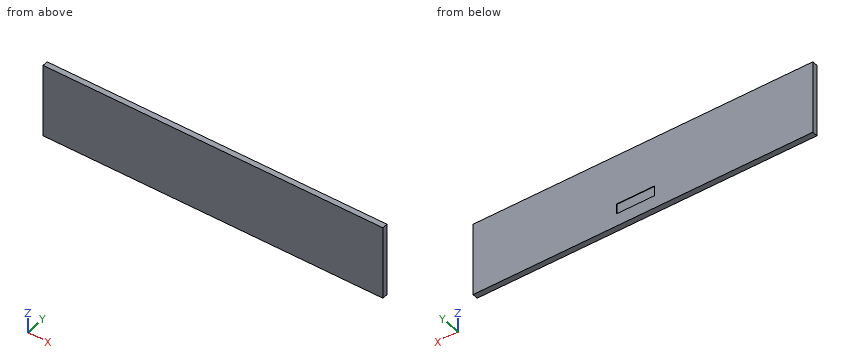
from build123d import *

# Parameters (mm, degrees)
SKETCH_1_W          = 1346
SKETCH_1_H          = 288
EXTRUDE_1_DEPTH     = 20
SHELL_1_T           = -2
SKETCH_2_W          = 1346
SKETCH_2_H          = 288
EXTRUDE_2_DEPTH     = 2
SKETCH_4_W          = 150
SKETCH_4_H          = 40
CUT_EXTRUDE_1_DEPTH = 2


with BuildPart() as part:
    # 草图1 → 凸台-拉伸1 (new body)
    with BuildSketch(Plane(origin=(0, 0, 0), x_dir=(1, 0, 0), z_dir=(0, 1, 0))):
        Rectangle(SKETCH_1_W, SKETCH_1_H)
    extrude(amount=-EXTRUDE_1_DEPTH)

    # 抽壳1
    shell_1_openings = [part.faces().sort_by_distance(p)[0] for p in [
        (0, -20, 0),
    ]]
    offset(amount=SHELL_1_T, openings=shell_1_openings, kind=Kind.INTERSECTION)

    # 草图2 → 凸台-拉伸2 (add)
    with BuildSketch(Plane.XZ.offset(20)):
        Rectangle(SKETCH_2_W, SKETCH_2_H)
    extrude(amount=EXTRUDE_2_DEPTH)

    # 草图4 → 切除-拉伸1 (cut)
    with BuildSketch(Plane(origin=(0, 0, 0), x_dir=(1, 0, 0), z_dir=(0, 1, 0))):
        with Locations((30, 74)):
            Rectangle(SKETCH_4_W, SKETCH_4_H)
    extrude(amount=-CUT_EXTRUDE_1_DEPTH, mode=Mode.SUBTRACT)


solid = part.part
Work out the finished part from the listing and answer in its coordinate system (mm). Give positions to 0.01 mm unless a question says otherwise; leave off trailing zeros. Order: outer loops, then holes, each group sorted by start corner. A loop starts at its lowest first (then second) coordinate and runs counter-clockwise, first axis right, second up. Notation, with made-up numbers: (4, -30.75) -> (60, -30.75) arc R21 ccw to (60, 8.25) -> close; hole circle Ø6 at (15.5, 7.5). An arc over 180 degrees is marked (long way). Answer as a JSON object with one key per item and string values. Group by question number.
1. Section B-B on z = 35 is taken. Determine the outline of the cut face in (x, y), plus the area to 3 significant figures.
2. Consider line 1 along X through (y, z) = (-12.75, 73.5); line 2 along Z through (x, y) = (589.5, -10.25); line 3 along Y through (x, z) = (-508, -84.5). Determine where each line is inside the solid, lowest interval first. Write a range as [from, to].
3. Section A-A on x = 583 is taken. Determine the outline of the cut face in (y, z), plus the area to 3 significant figures.
4. Section C-C on x = 41.5 is taken. Determine the outline of the cut face in (y, z).
Result sheet:
{
 "1": {"outline": "(-673, -22) -> (673, -22) -> (673, 0) -> (-673, 0) -> close; hole (-671, -20) -> (671, -20) -> (671, -2) -> (-671, -2) -> close", "area": "5,460 mm^2"},
 "2": {"line 1": "x = [-673, -671], [671, 673]", "line 2": "z = [-144, -142], [142, 144]", "line 3": "y = [-22, -20], [-2, 0]"},
 "3": {"outline": "(-22, -144) -> (0, -144) -> (0, 144) -> (-22, 144) -> close; hole (-20, -142) -> (-2, -142) -> (-2, 142) -> (-20, 142) -> close", "area": "1,220 mm^2"},
 "4": {"outline": "(-22, -144) -> (0, -144) -> (0, -94) -> (-2, -94) -> (-2, -142) -> (-20, -142) -> (-20, 142) -> (-2, 142) -> (-2, -54) -> (0, -54) -> (0, 144) -> (-22, 144) -> close"}
}
